Check sheet for the modelled part. Datum: model origin and axes. Units: mm. A direction names the side the tool comes from. Round coordinates to 2 decimals unless told otherwise and drop trailing zeros. Loops run counter-clockwise (first coordinate to the right, second up) from the corner with the lowest first, then second, coordinate; pieces in that order, holes last. Notation, with made-up numbers: M -27,-21 L -6,-21 A33 ccw -6,9 Z; hole C 89,3 d8. An arc over 180 degrees is marked long. Write item = value, one per line. Start each with the question number.
(1) Set-up check for faces 5 (the face through (-16.733, 25.07, 23.177)), 6 (the face through (1.099, 10.14, 20.024)): record each of +Z, -Z, +X, -X, +Y, -Y from which the full face is reachable in a straight line by a thin tool's end or side.
(2) Cross-section at C-C on y = 25.25. Record the boundary of the cut face in (x, z).
(3) Mould release check, pull along X, two halves, no side actions. Record for faces 1 (the face through (180, 15, 2)), 2 (the face through (-22.3, 20, 57.1)), 3 (the face through (-3, 15, -110)), 4 (the face through (-180, 15, 2)): pulls with the +X half, pulls with the -X half, needs draft (parallel to the pull), parting line crosses it, or undercut.
(4) Scan lines: L1, parallel to X at y = 24, z = 45; L2, parallel to X at y = 13.75, z = 45; L3, parallel to Z at x = -18, y = 23.75. Record each from-to range of solid material in increasing order. Write a range as from..to.
(5) Cross-section at B-B on x = 0. Record the boundary of the cut face in (y, z), plus the area to 3 significant figures.
(6) Cross-section at A-A on z = 45. Record the boundary of the cut face in (x, y), plus the area to 3 significant figures.
from build123d import *

# Parameters (mm, degrees)
SKETCH_1_W          = 360
SKETCH_1_H          = 220
EXTRUDE_1_DEPTH     = 30
SKETCH_2_R          = 27.5
CUT_EXTRUDE_1_DEPTH = 10
SKETCH_3_R          = 25
CUT_EXTRUDE_2_DEPTH = 214.072757527


with BuildPart() as part:
    # 草图1 → 凸台-拉伸1 (new body)
    with BuildSketch(Plane(origin=(0, 0, 0), x_dir=(1, 0, 0), z_dir=(0, 1, 0))):
        Rectangle(SKETCH_1_W, SKETCH_1_H)
    extrude(amount=EXTRUDE_1_DEPTH)

    # 草图2 → 切除-拉伸1 (cut)
    with BuildSketch(Plane(origin=(0, 30, 0), x_dir=(1, 0, 0), z_dir=(0, 1, 0))):
        with Locations(Location((0, -45, 0), (0, 0, 270))):
            Circle(SKETCH_2_R)
    extrude(amount=-CUT_EXTRUDE_1_DEPTH, mode=Mode.SUBTRACT)

    # 草图3 → 切除-拉伸2 (cut, through all)
    with BuildSketch(Plane(origin=(0, 30, 0), x_dir=(1, 0, 0), z_dir=(0, 1, 0))):
        with Locations(Location((0, -45, 0), (0, 0, 270))):
            Circle(SKETCH_3_R)
    extrude(amount=-CUT_EXTRUDE_2_DEPTH, mode=Mode.SUBTRACT)


solid = part.part
Result:
q1.face_5 = +Y
q1.face_6 = +Y, -Y
q2.outline = M -180,-110 L 180,-110 L 180,110 L -180,110 Z; hole C 0,45 d55
q3.face_1 = pulls with the +X half
q3.face_2 = undercut
q3.face_3 = needs draft
q3.face_4 = pulls with the -X half
q4.L1 = -180..-27.5, 27.5..180
q4.L2 = -180..-25, 25..180
q4.L3 = -110..24.21, 65.79..110
q5.outline = M 0,-110 L 30,-110 L 30,17.5 L 20,17.5 L 20,20 L 0,20 Z; M 0,70 L 20,70 L 20,72.5 L 30,72.5 L 30,110 L 0,110 Z
q5.area = 5,050 mm^2
q6.outline = M -180,0 L -25,0 L -25,20 L -27.5,20 L -27.5,30 L -180,30 Z; M 25,0 L 180,0 L 180,30 L 27.5,30 L 27.5,20 L 25,20 Z
q6.area = 9,250 mm^2
